```python
from build123d import *

# Parameters (mm, degrees)
BOSS_EXTRUDE1_DEPTH = 325
CUT_EXTRUDE1_DEPTH  = 330.772648957


with BuildPart() as part:
    # Sketch1 → Boss-Extrude1 (new, symmetric)
    with BuildSketch(Plane.XY):
        with BuildLine():
            Line((-17, -25), (17, -25))
            ThreePointArc((17, -25), (22.656854249, -22.656854249), (25, -17))
            Line((25, -17), (25, 17))
            ThreePointArc((25, 17), (22.656854249, 22.656854249), (17, 25))
            Line((17, 25), (-17, 25))
            ThreePointArc((-17, 25), (-22.656854249, 22.656854249), (-25, 17))
            Line((-25, 17), (-25, -17))
            ThreePointArc((-25, -17), (-22.656854249, -22.656854249), (-17, -25))
        make_face()
        with BuildLine():
            Line((-17, 21), (17, 21))
            ThreePointArc((17, 21), (19.828427125, 19.828427125), (21, 17))
            Line((21, 17), (21, -17))
            ThreePointArc((21, -17), (19.828427125, -19.828427125), (17, -21))
            Line((17, -21), (-17, -21))
            ThreePointArc((-17, -21), (-19.828427125, -19.828427125), (-21, -17))
            Line((-21, -17), (-21, 17))
            ThreePointArc((-21, 17), (-19.828427125, 19.828427125), (-17, 21))
        make_face(mode=Mode.SUBTRACT)
    extrude(amount=BOSS_EXTRUDE1_DEPTH, both=True)

    # Sketch2 → Cut-Extrude1 (cut, through all)
    with BuildSketch(Plane.ZY.offset(25)):
        Polygon((-325, 25), (-275, -25), (-325, -25), align=None)
    cut_extrude1 = extrude(amount=-CUT_EXTRUDE1_DEPTH, mode=Mode.SUBTRACT)

    # Mirror1: Cut-Extrude1 across plane
    add(cut_extrude1.mirror(Plane.XY), mode=Mode.SUBTRACT)


solid = part.part
```
The model under review builds one solid part; all positions refer to its coordinate system, in mm. A direction names the side the tool comes from. Round coordinates to 2 decimals unless told otherwise and drop trailing zeros. Order: outer loops, then holes, each group sorted by start corner. A loop starts at its lowest first (then second) coordinate and runs counter-clockwise, first axis right, second up. Notation, with made-up numbers: M 84,12.25 L 125,12.25 A31 ccw 125,43.25 Z; hole C -18,62 d7. An arc over 180 degrees is marked long. Use a Markdown table: item, result.
1) Consider section A-A (y = 1.5). Write out the cut boundary in (x, z).
Report:
| item | result |
|---|---|
| outline | M -25,-301.5 L -21,-301.5 L -21,301.5 L -25,301.5 Z; M 21,-301.5 L 25,-301.5 L 25,301.5 L 21,301.5 Z |
2) Draft analysis for pull direction X (two halves, no side actions). For faces 3 (the face through (25, 0, 4)), 4 (the face through (-25, 0, 4)), 5 (the face through (22, 0, -300)), 6 (the face through (21, 0, 4)), state which applies: released by +X, released by -X, zero draft, split by the parting line, or undercut.
Report:
| item | result |
|---|---|
| face 3 | released by +X |
| face 4 | released by -X |
| face 5 | zero draft |
| face 6 | undercut |
3) Wall thickness on line 1 along X through (y, z) = (4, 138); line 2 along Y through (x, z) = (-7, -288): over which ranges is each line inside the solid? List them lowest first. Write a range as [from, to].
Report:
| item | result |
|---|---|
| line 1 | [-25, -21], [21, 25] |
| line 2 | [21, 25] |
4) Insertion check: pin 1 (12 mm diameter, centred on x = -16, y = 15.5, fed in from -Z); pin 2 (2 mm diameter, centred on x = 19.5, z = 192, fed in from -Y); pin 3 (1.5 mm diameter, centred on x = -19.5, y = -5, fed in from +Z); pin 4 (12 mm diameter, centred on x = 20, z = -74.5, fed in from +Y). Each pin has a flat end and moves straight along its axis. Give the tip position at first contact, or say it passes through.
Report:
| item | result |
|---|---|
| pin 1 | z = -321.5 |
| pin 2 | y = -24.86 |
| pin 3 | through |
| pin 4 | y = 25 |
5) Consider section C-C (x = 6). Write out the cut boundary in (y, z).
Report:
| item | result |
|---|---|
| outline | M -25,-275 L -21,-279 L -21,279 L -25,275 Z; M 21,-321 L 25,-325 L 25,325 L 21,321 Z |
6) Tool access review of faces 1 (the face through (0, 21, 4)), 2 (the face through (0, 25, 5)): name each direction out of +Z, -Z, +X, -X, +Y, -Y from which nothing blocks a thin tool from reaching the whole face with its end or side.
Report:
| item | result |
|---|---|
| face 1 | +Z, -Z |
| face 2 | +Z, -Z, +X, -X, +Y |
7) Consider section B-B (z = 103.5). Write out the cut boundary in (x, y).
Report:
| item | result |
|---|---|
| outline | M -25,-17 A8 ccw -17,-25 L 17,-25 A8 ccw 25,-17 L 25,17 A8 ccw 17,25 L -17,25 A8 ccw -25,17 Z; hole M -21,-17 A4 ccw -17,-21 L 17,-21 A4 ccw 21,-17 L 21,17 A4 ccw 17,21 L -17,21 A4 ccw -21,17 Z |
